from build123d import *

# Parameters (mm, degrees)
SKETCH1_R           = 9
SKETCH1_R_2         = 2.5
BOSS_EXTRUDE1_DEPTH = 4
FILLET1_R           = 3


with BuildPart() as part:
    # Sketch1 → Boss-Extrude1 (new body)
    with BuildSketch(Plane(origin=(0, 0, 0), x_dir=(1, 0, 0), z_dir=(0, 1, 0))):
        Polygon((0, 0), (-80, 0), (-80, -75), (-15, -130), (0, -130), align=None)
        with Locations(Location((-57, -12, 0), (0, 0, 270))):
            Circle(SKETCH1_R, mode=Mode.SUBTRACT)
        with Locations(Location((-7.5, -122.5, 0), (0, 0, 270))):
            Circle(SKETCH1_R_2, mode=Mode.SUBTRACT)
        with BuildLine():
            Line((-25, -5), (-15, -5))
            ThreePointArc((-15, -5), (-10, -10), (-15, -15))
            Line((-15, -15), (-25, -15))
            ThreePointArc((-25, -15), (-30, -10), (-25, -5))
        make_face(mode=Mode.SUBTRACT)
        with BuildLine():
            Line((-65, -50), (-65, -60))
            ThreePointArc((-65, -60), (-70, -65), (-75, -60))
            Line((-75, -60), (-75, -50))
            ThreePointArc((-75, -50), (-70, -45), (-65, -50))
        make_face(mode=Mode.SUBTRACT)
        with BuildLine():
            Line((-45, -50), (-45, -60))
            ThreePointArc((-45, -60), (-50, -65), (-55, -60))
            Line((-55, -60), (-55, -50))
            ThreePointArc((-55, -50), (-50, -45), (-45, -50))
        make_face(mode=Mode.SUBTRACT)
    extrude(amount=BOSS_EXTRUDE1_DEPTH)

    # Fillet1
    fillet1_edges = [part.edges().sort_by_distance(p)[0] for p in [
        (0, 2, 130),
        (-15, 2, 130),
        (-80, 2, 75),
        (-80, 2, 0),
        (0, 2, 0),
    ]]
    fillet(fillet1_edges, radius=FILLET1_R)


solid = part.part
For this review, take the finished solid that the model builds, in its own axes (mm). A direction names the side the tool comes from. Coordinates: 2 decimals unless noted, no trailing zeros. Loops run counter-clockwise (first coordinate to the right, second up) from the corner with the lowest first, then second, coordinate; pieces in that order, holes last. Notation, with made-up numbers: (15, 7.25) -> (33, 7.25) arc R32 cw to (33, 42.25) -> close; hole circle Ø11 at (16, 45.5). An arc over 180 degrees is marked (long way). Write each question's results on one line, items separated by ' | '.
Q1. Add section C-C, the plane y = 0.9. State the section outline as (x, z) points, then the cut area to 3 significant figures.
Taken from the geometry:
outline: (-80, 3) arc R3 ccw to (-77, 0) -> (-3, 0) arc R3 ccw to (0, 3) -> (0, 127) arc R3 ccw to (-3, 130) -> (-13.9, 130) arc R3 ccw to (-15.84, 129.29) -> (-78.94, 75.9) arc R3 ccw to (-80, 73.61) -> close; hole (-75, 50) arc R5 ccw to (-65, 50) -> (-65, 60) arc R5 ccw to (-75, 60) -> close; hole circle Ø18 at (-57, 12); hole (-55, 50) arc R5 ccw to (-45, 50) -> (-45, 60) arc R5 ccw to (-55, 60) -> close; hole (-25, 5) -> (-15, 5) arc R5 ccw to (-15, 15) -> (-25, 15) arc R5 ccw to start; hole circle Ø5 at (-7.5, 122.5) | area: 7,800 mm²
Q2. Machinability: for faces 1 (the flat face through (-45, 2, 55)), 2 (the flat face through (-80, 2, 38)), which of the approach directions +Z, -Z, +X, -X, +Y, -Y give a long, thin tool a straight path to every point of the face, cutting with its end or side? Answer none if there is none.
Taken from the geometry:
face 1: +Y, -Y | face 2: +Z, -Z, -X, +Y, -Y
Q3. Mouldability with a two-part tool opening along Z and no side actions: class faces 3 (the flat face through (-47.83, 1.97, 102.22)), 4 (the flat face through (-39, 2, 0)), 5 (the cylindrical face through (-50, 2, 45)) as +Z half, -Z half, draft (parallel to the pull), parting line (faces both ways), or undercut.
Taken from the geometry:
face 3: +Z half | face 4: -Z half | face 5: undercut
Q4. Add section B-B, the plane z = 63. State the section outline as (x, y) points, then the cut area to 3 significant figures.
Taken from the geometry:
outline: (-80, 0) -> (-74, 0) -> (-74, 4) -> (-80, 4) -> close; (-66, 0) -> (-54, 0) -> (-54, 4) -> (-66, 4) -> close; (-46, 0) -> (0, 0) -> (0, 4) -> (-46, 4) -> close | area: 256 mm²
Q5. To check wall thickness, follow line 1 along X through (y, z) = (1.45, 54); line 2 along Z through (x, y) = (-54, 3.15); line 3 along X through (y, z) = (1.9, 12). State the ranges of each line that lie inside material, in increasing order. Write a range as [from, to].
Taken from the geometry:
line 1: [-80, -75], [-65, -55], [-45, 0] | line 2: [0, 3.51], [20.49, 47], [63, 97] | line 3: [-80, -66], [-48, -29.58], [-10.42, 0]
Q6. Add section D-D, the plane x = -50. State the section outline as (y, z) points, then the cut area to 3 significant figures.
Taken from the geometry:
outline: (0, 0) -> (4, 0) -> (4, 6.34) -> (0, 6.34) -> close; (0, 17.66) -> (4, 17.66) -> (4, 45) -> (0, 45) -> close; (0, 65) -> (4, 65) -> (4, 100.38) -> (0, 100.38) -> close | area: 276 mm²
Q7. For pin 1 Ø1 at (x, z) = (-59.5, 18.5) entering from +Y; pin 2 Ø2 at (x, y) = (-21, 1) entering from +Z, all flat-tipped, find the tip position at first contact; note any pin that passes through.
Taken from the geometry:
pin 1: through | pin 2: z = 125.77
Q8. Add section A-A, the plane x = -7.5. State the section outline as (y, z) points, then the cut area to 3 significant figures.
Taken from the geometry:
outline: (0, 0) -> (4, 0) -> (4, 120) -> (0, 120) -> close; (0, 125) -> (4, 125) -> (4, 130) -> (0, 130) -> close | area: 500 mm²
